Verification items for the finished model (mm, model axes). A direction names the side the tool comes from. Give positions to 0.01 mm unless a question says otherwise; leave off trailing zeros. Write each loop counter-clockwise with the first axis right and the second up, starting at its lowest first coordinate (ties: lowest second). Pieces come first, ordered by that corner, then holes. Notation, with made-up numbers: (21.25, 72.25) -> (38.25, 72.25) arc R15 cw to (38.25, 78.25) -> close; hole circle Ø8 at (36.5, 47). An arc over 180 degrees is marked (long way). Answer as CSV lines item,"result". Start each with the question number.
1) Gauge pin test, flat ends, axial feed: pin 1 Ø2 at (x, z) = (599.5, -12.5) entering from +Y; pin 2 Ø4.5 at (x, z) = (20, 0) entering from +Y; pin 3 Ø1.5 at (x, y) = (392, 10) entering from +Z. Record the tip position at first contact, or that the pin passes through.
2) Tool access check on faces 1 (the flat face through (659, 58, -10)), 2 (the flat face through (659, 58, 10)), 3 (the flat face through (659.14, 15.95, -9.21)). Record the directions out of +Z, -Z, +X, -X, +Y, -Y that give a thin tool (end or side, any length) a straight path to the whole face; none if there is none.
3) Material ranges on L1, parallel to Z at x = 1317, y = 82; L2, parallel to Y at x = 378.5, z = -1; L3, parallel to Z at x = 204.5, y = 40.5, recorded low to high.
4) Sectioned sample at B-B on y = 48. Record the cut outline in (x, z), and give its area (3 significant figures).
5) Sectioned sample at A-A on x = 491. Record the cut outline in (y, z).
```python
from build123d import *

# Parameters (mm, degrees)
EXTRUDE_1_DEPTH        = 1337
FILLET_1_R             = 1
HOLE_WIZARD_M6_1_D     = 5
HOLE_WIZARD_M6_1_DEPTH = 15
HOLE_WIZARD_M6_1_TIP   = 1.502151548


with BuildPart() as part:
    # 草图1 → 凸台-拉伸1 (new body)
    with BuildSketch(Plane(origin=(0, 0, 0), x_dir=(0, 0, -1), z_dir=(1, 0, 0))):
        Polygon((0, 0), (-17.320508076, 30), (-10, 30), (-10, 86), (10, 86), (10, 30), (17.320508076, 30), align=None)
    extrude(amount=EXTRUDE_1_DEPTH)

    # 圆角1
    fillet_1_edges = [part.edges().sort_by_distance(p)[0] for p in [
        (668.5, 0, 0),
    ]]
    fillet(fillet_1_edges, radius=FILLET_1_R)

    # M6 螺纹孔1
    with Locations(Plane(origin=(0, 86, 0), x_dir=(1, 0, 0), z_dir=(0, 1, 0))):
        with Locations((20, 0), (45, 0), (70, 0), (1317, 0), (1292, 0), (1267, 0)):
            Hole(HOLE_WIZARD_M6_1_D / 2, depth=HOLE_WIZARD_M6_1_DEPTH)
            with Locations((0, 0, -(HOLE_WIZARD_M6_1_DEPTH + HOLE_WIZARD_M6_1_TIP / 2))):  # 118° drill point
                Cone(0, HOLE_WIZARD_M6_1_D / 2, HOLE_WIZARD_M6_1_TIP, mode=Mode.SUBTRACT)


solid = part.part
```
Ans:
1,pin 1,"stops at y = 30"
1,pin 2,"stops at y = 70.85"
1,pin 3,"stops at z = 6.21"
2,face 1,"-Z, +X, -X, +Y"
2,face 2,"+Z, +X, -X, +Y"
2,face 3,"-Z, +X, -X, -Y"
3,L1,"z = -10 to -2.5, 2.5 to 10"
3,L2,"y = 1.73 to 86"
3,L3,"z = -10 to 10"
4,outline,"(0, -10) -> (1337, -10) -> (1337, 10) -> (0, 10) -> close"
4,area,"26,700 mm²"
5,outline,"(1.5, -0.87) -> (30, -17.32) -> (30, -10) -> (86, -10) -> (86, 10) -> (30, 10) -> (30, 17.32) -> (1.5, 0.87) arc R1 ccw to start"
